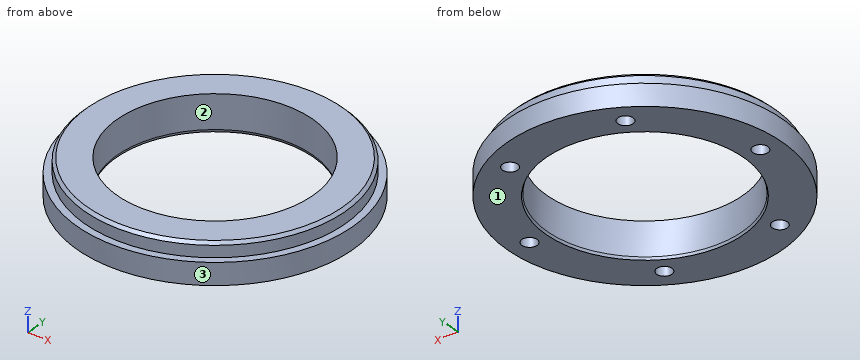
from build123d import *

# Parameters (mm, degrees)
SKETCH1_R                  = 95
SKETCH1_R_2                = 67.5
BOSS_EXTRUDE1_DEPTH        = 15
SKETCH2_R                  = 90
SKETCH2_R_2                = 67.5
BOSS_EXTRUDE2_DEPTH        = 10
CHAMFER1_SIZE              = 2
CHAMFER2_SIZE              = 1.8
CHAMFER2_SIZE2             = 0.655146422
M12X1_5_TAPPED_HOLE1_D     = 10.5
M12X1_5_TAPPED_HOLE1_DEPTH = 20
M12X1_5_TAPPED_HOLE1_TIP   = 3.15451825


with BuildPart() as part:
    # Sketch1 → Boss-Extrude1 (new body)
    with BuildSketch(Plane.XY):
        Circle(SKETCH1_R)
        Circle(SKETCH1_R_2, mode=Mode.SUBTRACT)
    extrude(amount=BOSS_EXTRUDE1_DEPTH)

    # Sketch2 → Boss-Extrude2 (add)
    with BuildSketch(Plane.XY.offset(15)):
        Circle(SKETCH2_R)
        Circle(SKETCH2_R_2, mode=Mode.SUBTRACT)
    extrude(amount=BOSS_EXTRUDE2_DEPTH)

    # Chamfer1
    chamfer1_edges = [part.edges().sort_by_distance(p)[0] for p in [
        (-90, 0, 25),
    ]]
    chamfer(chamfer1_edges, length=CHAMFER1_SIZE)

    # Chamfer2
    chamfer2_edges = [part.edges().sort_by_distance(p)[0] for p in [
        (-67.5, 0, 0),
    ]]
    chamfer2_side = [part.faces().sort_by_distance(p)[0] for p in [
        (-67.5, 0, 12.5),
    ]]
    chamfer(chamfer2_edges, length=CHAMFER2_SIZE, length2=CHAMFER2_SIZE2, reference=chamfer2_side[0])

    # M12x1.5 Tapped Hole1
    with Locations(Plane(origin=(40.25, 69.715045005, 0), x_dir=(-1, 0, 0), z_dir=(0, 0, -1))):
        with Locations((0, 0), (80.5, 0), (120.75, -69.715045005), (80.5, -139.43009001), (-40.25, -69.715045005), (0, -139.43009001)):
            Hole(M12X1_5_TAPPED_HOLE1_D / 2, depth=M12X1_5_TAPPED_HOLE1_DEPTH)
            with Locations((0, 0, -(M12X1_5_TAPPED_HOLE1_DEPTH + M12X1_5_TAPPED_HOLE1_TIP / 2))):  # 118° drill point
                Cone(0, M12X1_5_TAPPED_HOLE1_D / 2, M12X1_5_TAPPED_HOLE1_TIP, mode=Mode.SUBTRACT)


solid = part.part
Here's how the part is built. I have some questions about the finished solid (model axes, mm). Face numbers are marked on the shaded views. Coordinates: 2 decimals unless noted, no trailing zeros. Order: outer loops, then holes, each group sorted by start corner. A loop starts at its lowest first (then second) coordinate and runs counter-clockwise, first axis right, second up. Notation, with made-up numbers: M 30.5,20 L 88.5,20 A20 ccw 88.5,59 Z; hole C 67.25,81 d9. An arc over 180 degrees is marked long. Answer as CSV lines item,"result". Start each with the question number.
1. I want a section at A-A, the plane x = 0. Write out the boundary of the cut face in (y, z), and give its area (3 significant figures).
2. For pin 1 (6 mm diameter, centred on x = 64.5, z = 16.5, fed in from +Y); pin 2 (2 mm diameter, centred on x = -20, z = 3, fed in from -Y); pin 3 (8 mm diameter, centred on y = -10, z = 17.5, fed in from -X), each with a flat end and sliding along its axis, tell me the tip position at first contact or that it passes through.
3. We'd pull the mould along X, two halves only. Please class the marked faces 1, 2 and 3: released by +X, released by -X, zero draft, split by the parting line, or undercut.
4. I need wall thicknesses on line 1 (Y direction, x = -40.25, z = 11); line 2 (X direction, y = 46.5, z = 2.5); line 3 (X direction, y = -11, z = 16.75). Which ranges of each line are inside material? Lowest first, please. Write a range as [from, to].
5. I want a section at C-C, the plane z = 7. Write out the boundary of the cut face in (x, y), and give its area (3 significant figures).
6. I want a section at B-B, the plane z = 17.25. Write out the boundary of the cut face in (x, y).
Recorded:
1,outline,"M -95,0 L -68.16,0 L -67.5,1.8 L -67.5,25 L -88,25 L -90,23 L -90,15 L -95,15 Z; M 67.5,1.8 L 68.16,0 L 95,0 L 95,15 L 90,15 L 90,23 L 88,25 L 67.5,25 Z"
1,area,"1,270 mm2"
2,pin 1,"stops at y = 72.06"
2,pin 2,"stops at y = -93.08"
2,pin 3,"stops at x = -94.75"
3,face 1,"zero draft"
3,face 2,"undercut"
3,face 3,"split by the parting line"
4,line 1,"y = [-86.05, -74.97], [-64.47, -54.19], [54.19, 64.47], [74.97, 86.05]"
4,line 2,"x = [-82.84, -48.93], [48.93, 82.84]"
4,line 3,"x = [-89.33, -66.6], [66.6, 89.33]"
5,outline,"C 0,0 d190; hole C -80.5,0 d10.5; hole C 0,0 d135; hole C -40.25,-69.72 d10.5; hole C -40.25,69.72 d10.5; hole C 40.25,-69.72 d10.5; hole C 40.25,69.72 d10.5; hole C 80.5,0 d10.5"
5,area,"13,500 mm2"
6,outline,"C 0,0 d180; hole C -80.5,0 d10.5; hole C 0,0 d135; hole C -40.25,-69.72 d10.5; hole C -40.25,69.72 d10.5; hole C 40.25,-69.72 d10.5; hole C 40.25,69.72 d10.5; hole C 80.5,0 d10.5"
